The model under review builds one solid part; all positions refer to its coordinate system, in mm. A direction names the side the tool comes from. Give positions to 0.01 mm unless a question says otherwise; leave off trailing zeros. Order: outer loops, then holes, each group sorted by start corner. A loop starts at its lowest first (then second) coordinate and runs counter-clockwise, first axis right, second up. Notation, with made-up numbers: M 12,82 L 55,82 A21 cw 55,114 Z; hole C -15.5,25.25 d11. An arc over 180 degrees is marked long. One line per question, with ' | ' between items. Start each with the question number.
1. The part is to be moulded in two halves that separate along Z. For faces 4 (the face through (-1, 1, 4)), 5 (the face through (-65.3, 10.9, 3.9)), 6 (the face through (-28, 16, 8)), say which applies: +Z half, -Z half, draft (parallel to the pull), parting line (faces both ways), or undercut.
2. We need section B-B on x = -4.5. Write out the cut boundary in (y, z).
3. We need section D-D on x = -49. Write out the cut boundary in (y, z).
4. We need section A-A on y = 8. Write out the cut boundary in (x, z).
5. For faces 1 (the face through (-28, 16, 0)), 2 (the face through (-13.476, 5.121, 4.632)), 3 (the face through (-5.121, 36.636, 3.785)), list the 3-axis set-ups (+Z, -Z, +X, -X, +Y, -Y) from which the entire face can be reached by the end or side of a thin tool; tool diameter is ignored.
6. We need section C-C on z = 1.5. Write out the cut boundary in (x, y), then the cut area to 3 significant figures.
7. Wall thickness on L1, parallel to Y at x = -7.5, z = 4; L2, parallel to Z at x = -3, y = 35; L3, parallel to X at y = 5.5, z = 4: over which ranges is each line inside the solid? List them lowest first.
8. Insertion check: P1, Ø2, axis at y = 15, z = 4, coming from the +X side; P2, Ø1.5, axis at y = 33.5, z = 1.5, coming from the +X side; P3, Ø3, axis at x = -14, z = 3, coming from the +Y side; P4, Ø1, axis at y = 16, z = 1, coming from the -X side. Each pin has a flat end and moves straight along its axis. Give the tip position at first contact, or say it passes through.
```python
from build123d import *

# Parameters (mm, degrees)
EXTRUDE_1_DEPTH        = 8
HOLE_WIZARD_M4_2_D     = 3.3
HOLE_WIZARD_M4_2_DEPTH = 10.1
HOLE_WIZARD_M4_2_TIP   = 0.991420021
HOLE_WIZARD_M4_1_D     = 3.3
HOLE_WIZARD_M4_1_DEPTH = 10.1
HOLE_WIZARD_M4_1_TIP   = 0.991420021
CHAMFER_1_SIZE         = 2


with BuildPart() as part:
    # 草图1 → 凸台-拉伸1 (new body)
    with BuildSketch(Plane.XY):
        Polygon((0, 0), (0, 40), (-10, 40), (-70, 10), (-70, 0), align=None)
    extrude(amount=EXTRUDE_1_DEPTH)

    # M4 螺纹孔2
    with Locations(Plane(origin=(0, 0, 0), x_dir=(-1, 0, 0), z_dir=(0, -1, 0))):
        with Locations((15, -4), (65, -4)):
            Hole(HOLE_WIZARD_M4_2_D / 2, depth=HOLE_WIZARD_M4_2_DEPTH)
            with Locations((0, 0, -(HOLE_WIZARD_M4_2_DEPTH + HOLE_WIZARD_M4_2_TIP / 2))):  # 118° drill point
                Cone(0, HOLE_WIZARD_M4_2_D / 2, HOLE_WIZARD_M4_2_TIP, mode=Mode.SUBTRACT)

    # M4 螺纹孔1
    with Locations(Plane(origin=(0, 0, 0), x_dir=(0, 0, -1), z_dir=(1, 0, 0))):
        with Locations((-4, 35), (-4, 15)):
            Hole(HOLE_WIZARD_M4_1_D / 2, depth=HOLE_WIZARD_M4_1_DEPTH)
            with Locations((0, 0, -(HOLE_WIZARD_M4_1_DEPTH + HOLE_WIZARD_M4_1_TIP / 2))):  # 118° drill point
                Cone(0, HOLE_WIZARD_M4_1_D / 2, HOLE_WIZARD_M4_1_TIP, mode=Mode.SUBTRACT)

    # 倒角1
    chamfer_1_edges = [part.edges().sort_by_distance(p)[0] for p in [
        (0, 0, 4),
    ]]
    chamfer(chamfer_1_edges, length=CHAMFER_1_SIZE)


solid = part.part
```
Entries:
1) face 4: draft | face 5: undercut | face 6: +Z half
2) outline: M 0,0 L 40,0 L 40,8 L 0,8 Z; hole C 15,4 d3.3; hole C 35,4 d3.3
3) outline: M 0,0 L 20.5,0 L 20.5,8 L 0,8 Z
4) outline: M -70,0 L 0,0 L 0,8 L -70,8 Z; hole C -65,4 d3.3; hole C -15,4 d3.3
5) face 1: -Z, +X, -X, +Y, -Y | face 2: -Y | face 3: +X
6) outline: M -70,0 L -2,0 L 0,2 L 0,40 L -10,40 L -70,10 Z | area: 1,900 mm^2
7) L1: y = 0 to 13.35, 16.65 to 33.35, 36.65 to 40 | L2: z = 0 to 2.35, 5.65 to 8 | L3: x = -70 to -66.65, -63.35 to -16.65, -13.35 to 0
8) P1: stops at x = -10.49 | P2: stops at x = 0 | P3: stops at y = 38.75 | P4: stops at x = -59
